```python
from build123d import *

# Parameters (mm, degrees)
BASE_EXTRUDE_DEPTH = 33.02
SKETCH4_W          = 0.8
SKETCH4_H          = 22.495567884
CHAMFER_2_SIZE     = 2.4
FILLET_2_R         = 1


with BuildPart() as part:
    # Sketch1 → Base-Extrude (new body)
    with BuildSketch(Plane(origin=(0, 0, 0), x_dir=(0, 0, -1), z_dir=(1, 0, 0))):
        Polygon((28.575, 16.497783942), (28.575, -16.497783942), (0, -32.995567884), (-28.575, -16.497783942), (-28.575, 16.497783942), (0, 32.995567884), align=None)
    extrude(amount=BASE_EXTRUDE_DEPTH)

    # Sketch2 → Boss-Revolve1 (revolve)
    with BuildSketch(Plane.XY, mode=Mode.PRIVATE) as boss_revolve1_sk:
        Polygon((0, 0), (185.42, 0), (185.42, 13.8), (185.42, 19.05), (27.8072, 19.05), (0, 19.05), align=None)
    revolve(boss_revolve1_sk.sketch.rotate(Axis((0, 0, 0), (1, 0, 0)), 90), axis=Axis((0, 0, 0), (1, 0, 0)))

    # Sketch3 → Cut-Revolve1 (revolve, cut)
    with BuildSketch(Plane.XY):
        Polygon((0, 28.575), (5.438967404, 37.995567884), (5.438967404, 42.995567884), (-10, 42.995567884), (-10, 28.575), align=None)
    revolve(axis=Axis((0, 0, 0), (1, 0, 0)), mode=Mode.SUBTRACT)

    # Sketch4 → Cut-Revolve3 (revolve, cut)
    with BuildSketch(Plane.XY, mode=Mode.PRIVATE) as cut_revolve3_sk:
        with Locations((32.62, 31.747783942)):
            Rectangle(SKETCH4_W, SKETCH4_H)
    revolve(cut_revolve3_sk.sketch.rotate(Axis((0, 0, 0), (1, 0, 0)), 90), axis=Axis((0, 0, 0), (1, 0, 0)), mode=Mode.SUBTRACT)

    # Chamfer 2
    chamfer_2_edges = [part.edges().sort_by_distance(p)[0] for p in [
        (185.42, 0, -19.05),
    ]]
    chamfer(chamfer_2_edges, length=CHAMFER_2_SIZE)

    # Fillet 2
    fillet_2_edges = [part.edges().sort_by_distance(p)[0] for p in [
        (33.02, 0, -19.05),
    ]]
    fillet(fillet_2_edges, radius=FILLET_2_R)


solid = part.part
```
Part model, mm, in its own coordinate system. A direction names the side the tool comes from. Give positions to 0.01 mm unless a question says otherwise; leave off trailing zeros. Order: outer loops, then holes, each group sorted by start corner. A loop starts at its lowest first (then second) coordinate and runs counter-clockwise, first axis right, second up. Notation, with made-up numbers: (59.5, -34) - (113.5, -34) arc R23 cw to (113.5, -17) - close; hole circle Ø5 at (19, 3). An arc over 180 degrees is marked (long way). Use one line per item in the form item = value.
Item 1: Slice it at A-A on x = 18.5. Give the cut face in (y, z) (3 decimals), and give its area (3 significant figures).
Solution:
outline = (-32.996, 0) - (-16.498, -28.575) - (16.498, -28.575) - (32.996, 0) - (16.498, 28.575) - (-16.498, 28.575) - close
area = 2,830 mm2
Item 2: Probe probe 1 along X at (y, z) = (-12.5, 21.5); probe 2 along Z at (x, y) = (131, -15.5); probe 3 along Y at (x, z) = (12.5, -23.5). List the from-to ranges inside material, lowest first. Write a range as from..to.
Solution:
probe_1 = 0..32.22
probe_2 = -11.07..11.07
probe_3 = -19.43..19.43
Item 3: Slice it at B-B on x = 147.5. Give the cut face in (y, z).
Solution:
outline = circle Ø38.1 at (0, 0)
Item 4: Pin check, flat tips, straight feed: pin 1 Ø3 at (x, y) = (115, 3) entering from +Z; pin 2 Ø1.5 at (y, z) = (0, 21) entering from +X; pin 3 Ø10 at (x, z) = (21, -6.5) entering from +Y. Stop position of each tip, or through.
Solution:
pin_1 = 18.99
pin_2 = 33.02
pin_3 = 32.13
Item 5: Which spindle directions (+Z, -Z, +X, -X, +Y, -Y) get a long thin tool onto all of the face, cutting with end or side? Do faces 1 (the face through (16, 0, 28.575)), 2 (the face through (107.477, 18.597, -4.13)). Say none if no direction does.
Solution:
face_1 = +Z, +X, -X, +Y, -Y
face_2 = +X
